Source: CAD feature listing. Evaluate the final solid. Frame: model axes, mm. Round coordinates to 2 decimals unless told otherwise and drop trailing zeros. Order: outer loops, then holes, each group sorted by start corner. A loop starts at its lowest first (then second) coordinate and runs counter-clockwise, first axis right, second up. Notation, with made-up numbers: M 6,-7.75 L 25,-7.75 A25 cw 25,9.25 Z; hole C 50.5,23 d8. An arc over 180 degrees is marked long. Answer as CSV lines item,"result". Start each with the question number.
Item 1: Line query: line 1 (Z direction, x = 1958.5, y = 8.5); line 2 (Z direction, x = 281.5, y = -1.5); line 3 (Y direction, x = 729.5, z = -26). Output: solid intervals per line, ascending. Write a range as [from, to].
Item 2: Section query A-A on x = 1817. Return the cut outline in (y, z), plus the area to 3 significant figures.
Item 3: First-contact query: P1, Ø5.5, axis at x = 937.5, y = 9, coming from the -Z side; P2, Ø2, axis at x = 947.5, z = -29.5, coming from the +Y side. Flat tips, straight axial feed; report the tip coordinate or a pass-through.
from build123d import *

# Parameters (mm, degrees)
SKETCH_1_W             = 30
SKETCH_1_H             = 24
EXTRUDE_1_DEPTH        = 2200
CUT_EXTRUDE_1_DEPTH    = 2201.083862038
SKETCH_5_W             = 2200
SKETCH_5_H             = 3
EXTRUDE_2_DEPTH        = 22
CUT_EXTRUDE_2_DEPTH    = 22
PATTERN_LINEAR_1_COUNT = 6
PATTERN_LINEAR_1_PITCH = 510


with BuildPart() as part:
    # 草图1 → 凸台-拉伸1 (new body)
    with BuildSketch(Plane(origin=(0, 0, 0), x_dir=(0, 0, -1), z_dir=(1, 0, 0))):
        Rectangle(SKETCH_1_W, SKETCH_1_H)
    extrude(amount=EXTRUDE_1_DEPTH)

    # 草图2 → 切除-拉伸1 (cut, through all)
    with BuildSketch(Plane(origin=(2200, 0, 0), x_dir=(0, 0, -1), z_dir=(1, 0, 0))):
        Polygon((-6.2, 12), (-6.2, 0.7), (-8.5, 0.7), (-8.5, -3.9), (-3.5, -3.9), (-3.5, -5.5), (3.5, -5.5), (3.5, -3.9), (8.5, -3.9), (8.5, 0.7), (6.2, 0.7), (6.2, 12), align=None)
    extrude(amount=-CUT_EXTRUDE_1_DEPTH, mode=Mode.SUBTRACT)

    # 草图5 → 凸台-拉伸2 (add)
    with BuildSketch(Plane(origin=(0, 0, -15), x_dir=(-1, 0, 0), z_dir=(0, 0, -1))):
        with Locations((-1100, -10.5)):
            Rectangle(SKETCH_5_W, SKETCH_5_H)
    extrude(amount=EXTRUDE_2_DEPTH)

    # 草图6 → 切除-拉伸2 (cut)
    with BuildSketch(Plane.XZ.offset(12)):
        with BuildLine():
            Line((33.5, -22), (33.5, -30))
            ThreePointArc((33.5, -30), (30, -33.5), (26.5, -30))
            Line((26.5, -30), (26.5, -22))
            ThreePointArc((26.5, -22), (30, -18.5), (33.5, -22))
        make_face()
    cut_extrude_2 = extrude(amount=-CUT_EXTRUDE_2_DEPTH, mode=Mode.SUBTRACT)

    # 阵列(线性)1: 切除-拉伸2 ×6
    with Locations(*[(i * PATTERN_LINEAR_1_PITCH, 0, 0) for i in range(1, PATTERN_LINEAR_1_COUNT)]):
        add(cut_extrude_2, mode=Mode.SUBTRACT)


solid = part.part
Results:
1,line 1,"[-15, -6.2], [6.2, 15]"
1,line 2,"[-15, -8.5], [8.5, 15]"
1,line 3,"[-12, -9]"
2,outline,"M -12,-37 L -9,-37 L -9,-15 L 12,-15 L 12,-6.2 L 0.7,-6.2 L 0.7,-8.5 L -3.9,-8.5 L -3.9,-3.5 L -5.5,-3.5 L -5.5,3.5 L -3.9,3.5 L -3.9,8.5 L 0.7,8.5 L 0.7,6.2 L 12,6.2 L 12,15 L -12,15 Z"
2,area,"556 mm^2"
3,P1,"z = -15"
3,P2,"y = -9"
